```python
from build123d import *

# Parameters (mm, degrees)
SKETCH_1_W          = 28
SKETCH_1_H          = 28
EXTRUDE_1_DEPTH     = 106
SKETCH_2_R          = 2.6
CUT_EXTRUDE_1_DEPTH = 111.526015037
CUT_EXTRUDE_2_DEPTH = 111.526015037
CHAMFER_1_SIZE      = 1


with BuildPart() as part:
    # 草图1 → 凸台-拉伸1 (new body)
    with BuildSketch(Plane(origin=(0, 0, 0), x_dir=(1, 0, 0), z_dir=(0, 1, 0))):
        Rectangle(SKETCH_1_W, SKETCH_1_H)
    extrude(amount=EXTRUDE_1_DEPTH)

    # 草图2 → 切除-拉伸1 (cut, through all)
    with BuildSketch(Plane.XY.offset(14)):
        with Locations((0, 101)):
            Circle(SKETCH_2_R)
        with Locations((0, 53)):
            Circle(SKETCH_2_R)
        with Locations((0, 5)):
            Circle(SKETCH_2_R)
        with BuildLine():
            Line((-7, 60.5), (7, 60.5))
            ThreePointArc((7, 60.5), (9.121320344, 61.378679656), (10, 63.5))
            Line((10, 63.5), (10, 88))
            ThreePointArc((10, 88), (9.121320344, 90.121320344), (7, 91))
            Line((7, 91), (-7, 91))
            ThreePointArc((-7, 91), (-9.121320344, 90.121320344), (-10, 88))
            Line((-10, 88), (-10, 63.5))
            ThreePointArc((-10, 63.5), (-9.121320344, 61.378679656), (-7, 60.5))
        make_face()
        with BuildLine():
            Line((-7, 15), (7, 15))
            ThreePointArc((7, 15), (9.121320344, 15.878679656), (10, 18))
            Line((10, 18), (10, 42.5))
            ThreePointArc((10, 42.5), (9.121320344, 44.621320344), (7, 45.5))
            Line((7, 45.5), (-7, 45.5))
            ThreePointArc((-7, 45.5), (-9.121320344, 44.621320344), (-10, 42.5))
            Line((-10, 42.5), (-10, 18))
            ThreePointArc((-10, 18), (-9.121320344, 15.878679656), (-7, 15))
        make_face()
    extrude(amount=-CUT_EXTRUDE_1_DEPTH, mode=Mode.SUBTRACT)

    # 草图3 → 切除-拉伸2 (cut, through all)
    with BuildSketch(Plane(origin=(14, 0, 0), x_dir=(0, 0, -1), z_dir=(1, 0, 0))):
        with BuildLine():
            Line((-7, 60.5), (7, 60.5))
            ThreePointArc((7, 60.5), (9.121320344, 61.378679656), (10, 63.5))
            Line((10, 63.5), (10, 88))
            ThreePointArc((10, 88), (9.121320344, 90.121320344), (7, 91))
            Line((7, 91), (-7, 91))
            ThreePointArc((-7, 91), (-9.121320344, 90.121320344), (-10, 88))
            Line((-10, 88), (-10, 63.5))
            ThreePointArc((-10, 63.5), (-9.121320344, 61.378679656), (-7, 60.5))
        make_face()
        with BuildLine():
            Line((-7, 15), (7, 15))
            ThreePointArc((7, 15), (9.121320344, 15.878679656), (10, 18))
            Line((10, 18), (10, 42.5))
            ThreePointArc((10, 42.5), (9.121320344, 44.621320344), (7, 45.5))
            Line((7, 45.5), (-7, 45.5))
            ThreePointArc((-7, 45.5), (-9.121320344, 44.621320344), (-10, 42.5))
            Line((-10, 42.5), (-10, 18))
            ThreePointArc((-10, 18), (-9.121320344, 15.878679656), (-7, 15))
        make_face()
    extrude(amount=-CUT_EXTRUDE_2_DEPTH, mode=Mode.SUBTRACT)

    # 倒角1
    chamfer_1_edges = [part.edges().sort_by_distance(p)[0] for p in [
        (-14, 106, 0),
        (0, 106, 14),
        (14, 106, 0),
        (0, 0, 14),
        (-14, 0, 0),
        (0, 0, -14),
        (14, 0, 0),
        (14, 53, 14),
        (-14, 53, 14),
        (-14, 53, -14),
        (14, 53, -14),
        (0, 106, -14),
    ]]
    chamfer(chamfer_1_edges, length=CHAMFER_1_SIZE)


solid = part.part
```
The model under review builds one solid part; all positions refer to its coordinate system, in mm. A direction names the side the tool comes from. Give positions to 0.01 mm unless a question says otherwise; leave off trailing zeros. Write each loop counter-clockwise with the first axis right and the second up, starting at its lowest first coordinate (ties: lowest second). Pieces come first, ordered by that corner, then holes. Notation, with made-up numbers: M 30,19 L 34,19 A21 cw 34,52 Z; hole C 87,-13 d1. An arc over 180 degrees is marked long. Write item = value, one per line. Start each with the question number.
Q1. Clearance check with a flat-ended pin moving along its axis: pin 1 (3 mm diameter, centred on x = 0, y = 101, fed in from -Z). State where the tip first meets the part, or that it passes through.
Q2. We need section D-D (x = 0). State the section outline as (y, z) points.
Q3. Mouldability with a two-part tool opening along Z and no side actions: class faces 1 (the face through (-11.229, 44.938, -8.748)), 2 (the face through (0, 45.5, 0)), 3 (the face through (8.69, 61.02, -11.23)), 4 (the face through (-3, 52, -14)) as released by +Z, released by -Z, zero draft, split by the parting line, or undercut.
Q4. Machinability: for faces 5 (the face through (9.14, 44.6, 11.33)), 6 (the face through (0, 0, 0)), 7 (the face through (-11.229, 61.062, 8.748)), which of the approach directions +Z, -Z, +X, -X, +Y, -Y give a long, thin tool a straight path to every point of the face, cutting with its end or side? Answer none if there is none.
Q5. We need section C-C (y = 28). State the section outline as (x, z) points, plus the area to 3 significant figures.
Q6. We need section B-B (z = -0.25). State the section outline as (x, y) points, plus the area to 3 significant figures.
Q7. We need section A-A (y = 53). State the section outline as (x, z) points.
Q8. For line 1 (Y direction, x = 3.25, z = -11); line 2 (Y direction, x = -0.25, z = -7.5); line 3 (Z direction, x = 12, y = 24), list the stretches that pass through material, from the lowest coordinate up.
Result set:
q1.pin_1 = through
q2.outline = M 0,-13 L 1,-14 L 2.4,-14 L 2.4,14 L 1,14 L 0,13 Z; M 7.6,-14 L 15,-14 L 15,14 L 7.6,14 Z; M 45.5,-14 L 50.4,-14 L 50.4,14 L 45.5,14 Z; M 55.6,-14 L 60.5,-14 L 60.5,14 L 55.6,14 Z; M 91,-14 L 98.4,-14 L 98.4,14 L 91,14 Z; M 103.6,-14 L 105,-14 L 106,-13 L 106,13 L 105,14 L 103.6,14 Z
q3.face_1 = undercut
q3.face_2 = undercut
q3.face_3 = zero draft
q3.face_4 = released by -Z
q4.face_5 = +Z, -Z
q4.face_6 = +Z, -Z, +X, -X, -Y
q4.face_7 = +X, -X
q5.outline = M -14,-13 L -13,-14 L -10,-14 L -10,-10 L -14,-10 Z; M -14,10 L -10,10 L -10,14 L -13,14 L -14,13 Z; M 10,-14 L 13,-14 L 14,-13 L 14,-10 L 10,-10 Z; M 10,10 L 14,10 L 14,13 L 13,14 L 10,14 Z
q5.area = 62.0 mm2
q6.outline = M -14,1 L -13,0 L 13,0 L 14,1 L 14,15 L -14,15 Z; M -14,45.5 L 14,45.5 L 14,60.5 L -14,60.5 Z; M -14,91 L 14,91 L 14,105 L 13,106 L -13,106 L -14,105 Z; hole C 0,5 d5.2; hole C 0,53 d5.2; hole C 0,101 d5.2
q6.area = 1,190 mm2
q7.outline = M -14,-13 L -13,-14 L -2.6,-14 L -2.6,14 L -13,14 L -14,13 Z; M 2.6,-14 L 13,-14 L 14,-13 L 14,13 L 13,14 L 2.6,14 Z
q8.line_1 = 0 to 15, 45.5 to 60.5, 91 to 106
q8.line_2 = 0 to 2.41, 7.59 to 15, 45.5 to 50.41, 55.59 to 60.5, 91 to 98.41, 103.59 to 106
q8.line_3 = -14 to -10, 10 to 14
